from build123d import *

# Parameters (mm, degrees)
SKETCH1_R                    = 72
BOSS_EXTRUDE1_DEPTH          = 58
SKETCH2_R                    = 55
BOSS_EXTRUDE2_DEPTH          = 5
F_10_5_10_5_DIAMETER_HOLE1_D = 10.5
SKETCH5_R                    = 55
CUT_EXTRUDE1_DEPTH           = 42
SKETCH6_R                    = 30.25
CUT_EXTRUDE2_DEPTH           = 5
SKETCH7_R                    = 40
CUT_EXTRUDE3_DEPTH           = 12
SKETCH9_R                    = 50
CUT_EXTRUDE4_DEPTH           = 4


with BuildPart() as part:
    # Sketch1 → Boss-Extrude1 (new body)
    with BuildSketch(Plane.XY):
        with Locations(Location((0, 0, 0), (0, 0, 180))):
            Circle(SKETCH1_R)
    extrude(amount=BOSS_EXTRUDE1_DEPTH)

    # Sketch2 → Boss-Extrude2 (add)
    with BuildSketch(Plane.XY.offset(58)):
        Circle(SKETCH2_R)
    extrude(amount=BOSS_EXTRUDE2_DEPTH)

    # Ø10.5 (10.5) Diameter Hole1 (through all)
    with Locations(Plane(origin=(0, 0, 0), x_dir=(-1, 0, 0), z_dir=(0, 0, -1))):
        with Locations((-11.113483371, 63.027696193), (11.113483371, 63.027696193), (49.02684436, 41.13840702), (60.14032773, 21.889289173), (60.14032773, -21.889289173), (49.02684436, -41.13840702), (11.113483371, -63.027696193), (-11.113483371, -63.027696193), (-49.02684436, -41.13840702), (-60.14032773, -21.889289173), (-60.14032773, 21.889289173), (-49.02684436, 41.13840702)):
            Hole(F_10_5_10_5_DIAMETER_HOLE1_D / 2)

    # Sketch5 → Cut-Extrude1 (cut)
    with BuildSketch(Plane(origin=(0, 0, 0), x_dir=(-1, 0, 0), z_dir=(0, 0, -1))):
        with Locations(Location((0, 0, 0), (0, 0, 180))):
            Circle(SKETCH5_R)
    extrude(amount=-CUT_EXTRUDE1_DEPTH, mode=Mode.SUBTRACT)

    # Sketch6 → Cut-Extrude2 (cut)
    with BuildSketch(Plane(origin=(0, 0, 42), x_dir=(-1, 0, 0), z_dir=(0, 0, -1))):
        Circle(SKETCH6_R)
    extrude(amount=-CUT_EXTRUDE2_DEPTH, mode=Mode.SUBTRACT)

    # Sketch7 → Cut-Extrude3 (cut)
    with BuildSketch(Plane(origin=(0, 0, 47), x_dir=(-1, 0, 0), z_dir=(0, 0, -1))):
        Circle(SKETCH7_R)
    extrude(amount=-CUT_EXTRUDE3_DEPTH, mode=Mode.SUBTRACT)

    # Sketch9 → Cut-Extrude4 (cut)
    with BuildSketch(Plane(origin=(0, 0, 59), x_dir=(-1, 0, 0), z_dir=(0, 0, -1))):
        Circle(SKETCH9_R)
    extrude(amount=-CUT_EXTRUDE4_DEPTH, mode=Mode.SUBTRACT)


solid = part.part
Verification items for the finished model (mm, model axes). A direction names the side the tool comes from. Give positions to 0.01 mm unless a question says otherwise; leave off trailing zeros. Write each loop counter-clockwise with the first axis right and the second up, starting at its lowest first coordinate (ties: lowest second). Pieces come first, ordered by that corner, then holes. Notation, with made-up numbers: (54.25, 32.5) - (72.25, 32.5) arc R31 cw to (72.25, 61.5) - close; hole circle Ø4 at (39.25, 5). An arc over 180 degrees is marked (long way). Answer as CSV lines item,"result". Start each with the question number.
1. Sectioned sample at A-A (y = 0). Record the boundary of the cut face in (x, z).
2. Sectioned sample at C-C (z = 21). Count the separate pieces of the cut face and the enclosed holes in it, then the cut area to 3 significant figures.
3. Thickness scan on line 1 (X direction, y = 44, z = 6); line 2 (Y direction, x = 48, z = 47.5); line 3 (Y direction, x = -9, z = 21). Record the ranges inside material, lowest first.
4. Draft check along Y on faces 1 (the face through (-11.923, -53.692, 60.465)), 2 (the face through (10.43, -57.822, 29.406)), 3 (the face through (12, -49, 63)). Enter one of: pulls with the +Y half, pulls with the -Y half, needs draft (parallel to the pull), parting line crosses it, or undercut.
5. Set-up check for faces 4 (the face through (24, 24, 42)), 5 (the face through (8.67, -39.05, 52.92)), 6 (the face through (-8.29, -58.6, 29.41)): record each of +Z, -Z, +X, -X, +Y, -Y from which the full face is reachable in a straight line by a thin tool's end or side.
6. Sectioned sample at D-D (x = 58). Record the boundary of the cut face in (y, z), then the cut area to 3 significant figures.
7. Depth check by flat-ended pin: pin 1 (12 mm diameter, centred on y = 27, z = 34.5, fed in from -X); pin 2 (2 mm diameter, centred on x = -2, z = 15, fed in from -Y); pin 3 (3 mm diameter, centred on y = 32.5, z = 43, fed in from -X). Enter the tip coordinate at first touch or a pass-through.
Derived:
1,outline,"(-72, 0) - (-55, 0) - (-55, 42) - (-30.25, 42) - (-30.25, 47) - (-40, 47) - (-40, 59) - (-50, 59) - (-50, 63) - (-55, 63) - (-55, 58) - (-72, 58) - close; (30.25, 42) - (55, 42) - (55, 0) - (72, 0) - (72, 58) - (55, 58) - (55, 63) - (50, 63) - (50, 59) - (40, 59) - (40, 47) - (30.25, 47) - close"
2,separate pieces,"1"
2,enclosed holes,"13"
2,area,"5,740 mm²"
3,line 1,"-56.99 to -53.43, -44.63 to -33, 33 to 44.63, 53.43 to 56.99"
3,line 2,"-53.67 to -46.29, -35.99 to 35.99, 46.29 to 53.67"
3,line 3,"-71.44 to -67.83, -58.22 to -54.26, 54.26 to 58.22, 67.83 to 71.44"
4,face 1,"parting line crosses it"
4,face 2,"undercut"
4,face 3,"needs draft"
5,face 4,"-Z"
5,face 5,"+Z"
5,face 6,"+Z, -Z"
6,outline,"(-42.66, 0) - (-26.68, 0) - (-26.68, 58) - (-42.66, 58) - close; (-17.1, 0) - (17.1, 0) - (17.1, 58) - (-17.1, 58) - close; (26.68, 0) - (42.66, 0) - (42.66, 58) - (26.68, 58) - close"
6,area,"3,840 mm²"
7,pin 1,"x = -68.87"
7,pin 2,"y = -71.99"
7,pin 3,"x = -64.98"
